Design review of the part built by this model. Coordinates are the model's own, in mm. Coordinates: 2 decimals unless noted, no trailing zeros. Loops run counter-clockwise (first coordinate to the right, second up) from the corner with the lowest first, then second, coordinate; pieces in that order, holes last. Notation, with made-up numbers: (33, 47.25) - (92, 47.25) arc R16 ccw to (92, 60.25) - close; hole circle Ø1 at (-7.75, 19.25). An arc over 180 degrees is marked (long way). One line per question, with ' | ' between items.
from build123d import *

# Parameters (mm, degrees)
SKETCH1_R           = 259.5
SKETCH1_R_2         = 210.5
BOSS_EXTRUDE1_DEPTH = 1
CUT_EXTRUDE1_REACH  = 368.99
SKETCH2_R           = 11.5
CIRPATTERN1_COUNT   = 6


with BuildPart() as part:
    # Sketch1 → Boss-Extrude1 (new body)
    with BuildSketch(Plane.XY):
        Circle(SKETCH1_R)
        Circle(SKETCH1_R_2, mode=Mode.SUBTRACT)
    extrude(amount=BOSS_EXTRUDE1_DEPTH)

    # Sketch2 → Cut-Extrude1 (cut, up to next)
    with BuildSketch(Plane.XY.offset(1), mode=Mode.PRIVATE) as cut_extrude1_sk1:
        with Locations((-235, 0)):
            Circle(SKETCH2_R)
    cut_extrude1_tool1 = extrude(cut_extrude1_sk1.sketch, amount=-CUT_EXTRUDE1_REACH, mode=Mode.PRIVATE) & part.part
    cut_extrude1 = cut_extrude1_tool1.solids().sort_by_distance((-235, 0, 1))[0]
    add(cut_extrude1, mode=Mode.SUBTRACT)

    # CirPattern1: Cut-Extrude1 ×6 about axis
    cirpattern1_axis = Axis((0, 0, 0), (0, 0, 1))
    for i in range(1, CIRPATTERN1_COUNT):
        add(cut_extrude1.rotate(cirpattern1_axis, i * 360 / CIRPATTERN1_COUNT), mode=Mode.SUBTRACT)


solid = part.part
Q1. Draft analysis for pull direction Y (two halves, no side actions). For faces 1 (the cylindrical face through (109.024, 211.288, 0.507)), 2 (the flat face through (-20, -210, 0)), 3 (the cylindrical face through (247.517, 77.947, 0.493)), state which applies: +Y half, -Y half, draft (parallel to the pull), parting line (faces both ways), or undercut.
Returned:
face 1: undercut | face 2: draft | face 3: parting line
Q2. For pin 1 (14 mm diameter, centred on x = -117.5, y = -203.52, fed in from -Z), flat-tipped, find the tip position at first contact; note if it passes through.
Returned:
pin 1: passes through
Q3. To check wall thickness, follow line 1 along Y through (x, z) = (-52, 0.6); line 2 along Y through (x, z) = (-161.5, 0.9); line 3 along X through (y, z) = (29, 0.3). State the ranges of each line that lie inside material, in increasing order.
Returned:
line 1: y = -254.24 to -203.98, 203.98 to 254.24 | line 2: y = -203.12 to -135.01, 135.01 to 203.12 | line 3: x = -257.87 to -208.49, 208.49 to 257.87
Q4. Take a section at A-A (x = 0). Give the boundary of the cut face in (y, z), plus the area to 3 significant figures.
Returned:
outline: (-259.5, 0) - (-210.5, 0) - (-210.5, 1) - (-259.5, 1) - close; (210.5, 0) - (259.5, 0) - (259.5, 1) - (210.5, 1) - close | area: 98.0 mm²
Q5. Take a section at C-C (z = 0.4). Give the boundary of the cut face in (x, y).
Returned:
outline: circle Ø519 at (0, 0); hole circle Ø23 at (-235, 0); hole circle Ø421 at (0, 0); hole circle Ø23 at (-117.5, -203.52); hole circle Ø23 at (-117.5, 203.52); hole circle Ø23 at (117.5, -203.52); hole circle Ø23 at (117.5, 203.52); hole circle Ø23 at (235, 0)
Q6. Take a section at B-B (y = -162). Give the boundary of the cut face in (x, z).
Returned:
outline: (-202.72, 0) - (-134.41, 0) - (-134.41, 1) - (-202.72, 1) - close; (134.41, 0) - (202.72, 0) - (202.72, 1) - (134.41, 1) - close
